```python
from build123d import *

# Parameters (mm, degrees)
EXTRUDE_1_DEPTH     = 260
SKETCH_2_W          = 50
SKETCH_2_H          = 15
CUT_EXTRUDE_1_DEPTH = 10


with BuildPart() as part:
    # 草图1 → 凸台-拉伸1 (new body)
    with BuildSketch(Plane.XY):
        Polygon((0, 0), (70, 0), (70, -8), (8, -8), (8, -30), (0, -30), align=None)
    extrude(amount=EXTRUDE_1_DEPTH)

    # 草图2 → 切除-拉伸1 (cut)
    with BuildSketch(Plane.ZY):
        with Locations((185, -22.5)):
            Rectangle(SKETCH_2_W, SKETCH_2_H)
    extrude(amount=-CUT_EXTRUDE_1_DEPTH, mode=Mode.SUBTRACT)


solid = part.part
```
Verification items for the finished model (mm, model axes). A direction names the side the tool comes from. Coordinates: 2 decimals unless noted, no trailing zeros. Loops run counter-clockwise (first coordinate to the right, second up) from the corner with the lowest first, then second, coordinate; pieces in that order, holes last. Notation, with made-up numbers: (13.5, 56.5) -> (17.5, 56.5) arc R17 ccw to (17.5, 69.5) -> close; hole circle Ø2 at (-25, 12). An arc over 180 degrees is marked (long way). Answer in a Markdown table with one row per item. Add a question column.
1. Draft check along Z on faces 4 (the face through (30, -7, 260)), 5 (the face through (30, -7, 0)), 6 (the face through (4, -23, 160)). Enter one of: +Z half, -Z half, draft (parallel to the pull), parting line (faces both ways), or undercut.
2. Section check A-A, the plane y = -19.25. Enter the section's corners in (x, z), then the cut area to 3 significant figures.
3. Section check B-B, the plane z = 99.5. Enter the section's corners in (x, y), then the cut area to 3 significant figures.
4. Material ranges on probe 1 along Z at (x, y) = (6.5, -20.25); probe 2 along Y at (x, z) = (62, 20); probe 3 along X at (y, z) = (-15.5, 66), recorded low to high. Write a range as [from, to].
5. Access from +Z, -Z, +X, -X, +Y, -Y to the whole of each face (thin tool, end or side, straight path). Record for faces 1 (the face through (39, -8, 128)), 2 (the face through (70, -4, 128)), 3 (the face through (4, -15, 185)).
6. Depth check by flat-ended pin: P1, Ø9, axis at x = 3.5, z = 181, coming from the -Y side; P2, Ø6, axis at y = -22.5, z = 217, coming from the +X side; P3, Ø12, axis at x = 30, y = -19, coming from the +Z side. Enter the tip coordinate at first touch or a pass-through.
7. Section check C-C, the plane x = 17.5. Enter the section's corners in (y, z), then the cut area to 3 significant figures.
Derived:
| question | item | result |
|---|---|---|
| 1 | face 4 | +Z half |
| 1 | face 5 | -Z half |
| 1 | face 6 | undercut |
| 2 | outline | (0, 0) -> (8, 0) -> (8, 160) -> (0, 160) -> close; (0, 210) -> (8, 210) -> (8, 260) -> (0, 260) -> close |
| 2 | area | 1,680 mm² |
| 3 | outline | (0, -30) -> (8, -30) -> (8, -8) -> (70, -8) -> (70, 0) -> (0, 0) -> close |
| 3 | area | 736 mm² |
| 4 | probe 1 | z = [0, 160], [210, 260] |
| 4 | probe 2 | y = [-8, 0] |
| 4 | probe 3 | x = [0, 8] |
| 5 | face 1 | +Z, -Z, +X, -Y |
| 5 | face 2 | +Z, -Z, +X, +Y, -Y |
| 5 | face 3 | +X, -X, -Y |
| 6 | P1 | stops at y = -15 |
| 6 | P2 | stops at x = 8 |
| 6 | P3 | passes through |
| 7 | outline | (-8, 0) -> (0, 0) -> (0, 260) -> (-8, 260) -> close |
| 7 | area | 2,080 mm² |
